```python
from build123d import *

# Parameters (mm, degrees)
SKETCH_1_R               = 6
EXTRUDE_1_DEPTH          = 10
CUT_EXTRUDE_2_DEPTH      = 18.62337463
PATTERN_CIRCULAR_1_COUNT = 3
SKETCH_2_R               = 7.375
SKETCH_2_R_2             = 6
EXTRUDE_2_DEPTH          = 1.4
SKETCH_4_OUTSIDE_W       = 166.146
SKETCH_4_OUTSIDE_H       = 169.086
SKETCH_4_OUTSIDE_R       = 9.5
CUT_EXTRUDE_3_DEPTH      = 18.62337463
CUT_EXTRUDE_3_DRAFT      = -75
SKETCH_5_R               = 7.535
CUT_EXTRUDE_4_DEPTH      = 0.2


with BuildPart() as part:
    # 草图1 → 拉伸1 (new body)
    with BuildSketch(Plane.XY):
        Polygon((0, 10.969655115), (-9.5, 5.484827557), (-9.5, -5.484827557), (0, -10.969655115), (9.5, -5.484827557), (9.5, 5.484827557), align=None)
        Circle(SKETCH_1_R, mode=Mode.SUBTRACT)
    extrude(amount=EXTRUDE_1_DEPTH)

    # 草图3 → 切除-拉伸2 (cut, symmetric)
    with BuildSketch(Plane(origin=(0, 0, 0), x_dir=(0, 0, -1), z_dir=(1, 0, 0))):
        Polygon((-9.4, 9.540494522), (-8.6, 9.167448395), (-8.6, 0), (-10, 0), (-10, 10.969655115), (-9.4, 10.969655115), align=None)
    cut_extrude_2 = extrude(amount=CUT_EXTRUDE_2_DEPTH, both=True, mode=Mode.SUBTRACT)

    # 阵列(圆周)1: 切除-拉伸2 ×3 about axis
    pattern_circular_1_axis = Axis((0, 0, 0), (0, 0, 1))
    for i in range(1, PATTERN_CIRCULAR_1_COUNT):
        add(cut_extrude_2.rotate(pattern_circular_1_axis, i * 360 / PATTERN_CIRCULAR_1_COUNT), mode=Mode.SUBTRACT)

    # 草图2 → 拉伸2 (add)
    with BuildSketch(Plane.XY.offset(8.6)):
        with Locations(Location((0, 0, 0), (0, 0, 180))):
            Circle(SKETCH_2_R)
        Circle(SKETCH_2_R_2, mode=Mode.SUBTRACT)
    extrude(amount=EXTRUDE_2_DEPTH)


with BuildPart() as cut_extrude_3_tool:
    # 草图4 outside → 切除-拉伸3 (with draft: the straight prism first)
    with BuildSketch(Plane(origin=(0, 0, 0), x_dir=(-1, 0, 0), z_dir=(0, 0, -1))):
        Rectangle(SKETCH_4_OUTSIDE_W, SKETCH_4_OUTSIDE_H)
        Circle(SKETCH_4_OUTSIDE_R, mode=Mode.SUBTRACT)
    extrude(amount=-CUT_EXTRUDE_3_DEPTH)
    # 切除-拉伸3: the draft: its side faces are tilted about the plane it starts from
    cut_extrude_3_sides = [cut_extrude_3_tool.faces().sort_by_distance(p)[0] for p in [
        (0, -84.543, 9.311687315),
        (-83.073, 0, 9.311687315),
        (0, 84.543, 9.311687315),
        (83.073, 0, 9.311687315),
        (9.5, 0, 9.311687315),
    ]]
    draft(cut_extrude_3_sides, Plane(origin=(0, 0, 0), x_dir=(-1, 0, 0), z_dir=(0, 0, -1)), CUT_EXTRUDE_3_DRAFT)


with BuildPart() as part_1:
    add(part.part)

    # 切除-拉伸3: cut by cut_extrude_3_tool
    add(cut_extrude_3_tool.part, mode=Mode.SUBTRACT)

    # 草图5 → 切除-拉伸4 (cut)
    with BuildSketch(Plane(origin=(0, 0, 0), x_dir=(-1, 0, 0), z_dir=(0, 0, -1))):
        Circle(SKETCH_5_R)
    extrude(amount=-CUT_EXTRUDE_4_DEPTH, mode=Mode.SUBTRACT)


solid = part_1.part
```
The listing builds one solid part. Answer for the finished solid, in the listing's coordinates (mm). A direction names the side the tool comes from. Give positions to 0.01 mm unless a question says otherwise; leave off trailing zeros. Order: outer loops, then holes, each group sorted by start corner. A loop starts at its lowest first (then second) coordinate and runs counter-clockwise, first axis right, second up. Notation, with made-up numbers: (15.25, 38) -> (58.25, 38) arc R7 cw to (58.25, 42) -> close; hole circle Ø9 at (74, -28.5). An arc over 180 degrees is marked (long way). Answer as CSV lines item,"result". Start each with the question number.
Q1. Find the intervals of material crossed by L1, parallel to X at y = 0, z = 5; L2, parallel to Z at x = -6.75, y = -2; L3, parallel to X at y = 5.25, z = 3, in increasing order.
Q2. Determine the mould class of faces 1 (the flat face through (0, 10, 9.4)), 2 (the cylindrical face through (-6, 0, 5)), 3 (the cylindrical face through (-7.034, -2.215, 9.29)), 4 (the flat face through (4.8, 8.2, 4.6)) for opening direction X: pulls with the +X half, pulls with the -X half, needs draft (parallel to the pull), parting line crosses it, or undercut.
Q3. Which of the six approach directions +Z, -Z, +X, -X, +Y, -Y give full straight-line access (tool end or side, diameter ignored) to faces 5 (the flat face through (9.5, 0, 5)), 6 (the flat face through (6, -2, 0.2)), 7 (the flat face through (0.04, 9.36, 9.01)), 8 (the flat face through (8.08, -4.72, 9.01))?
Q4. A cutting plane is placed at A-A (z = 2.25). Determine the outline of the cut face in (x, y).
Q5. Given pin 1 (7 mm diameter, centred on x = 0, y = 0, fed in from +Z); pin 2 (9.5 mm diameter, centred on x = 2, y = -5.5, fed in from +Z); pin 3 (1 mm diameter, centred on x = -5.5, y = -1.5, fed in from -Z); pin 4 (2.5 mm diameter, centred on x = 8.5, y = -5, fed in from +Z), each flat-ended and moving along its own axis, determine where each tip first touches the part or whether it passes through.
Results found:
1,L1,"-9.5 to -6, 6 to 9.5"
1,L2,"0.2 to 10"
1,L3,"-9.5 to -2.9, 2.9 to 9.5"
2,face 1,"needs draft"
2,face 2,"undercut"
2,face 3,"undercut"
2,face 4,"pulls with the +X half"
3,face 5,"+Z, -Z, +X, +Y, -Y"
3,face 6,"-Z"
3,face 7,"+Z, +X, -X"
3,face 8,"+Z"
4,outline,"(-9.5, -5.48) -> (0, -10.97) -> (9.5, -5.48) -> (9.5, 5.48) -> (0, 10.97) -> (-9.5, 5.48) -> close; hole circle Ø12 at (0, 0)"
5,pin 1,"through"
5,pin 2,"z = 10"
5,pin 3,"z = 0.2"
5,pin 4,"z = 9.4"
